from build123d import *

# Parameters (mm, degrees)
BOSS_EXTRUDE1_DEPTH = 10
SKETCH2_R           = 10
CUT_EXTRUDE1_DEPTH  = 140.306317158


with BuildPart() as part:
    # Sketch1 → Boss-Extrude1 (new body)
    with BuildSketch(Plane.XY):
        with BuildLine():
            Line((-117.5, 20), (117.5, 20))
            ThreePointArc((117.5, 20), (137.5, 0), (117.5, -20))
            Line((117.5, -20), (-117.5, -20))
            ThreePointArc((-117.5, -20), (-137.5, 0), (-117.5, 20))
        make_face()
    extrude(amount=BOSS_EXTRUDE1_DEPTH)

    # Sketch2 → Cut-Extrude1 (cut, through all)
    with BuildSketch(Plane.XY.offset(10)):
        with Locations((-117.5, 0)):
            Circle(SKETCH2_R)
        with Locations((117.5, 0)):
            Circle(SKETCH2_R)
    extrude(amount=-CUT_EXTRUDE1_DEPTH, mode=Mode.SUBTRACT)


solid = part.part
The model under review builds one solid part; all positions refer to its coordinate system, in mm. Give positions to 0.01 mm unless a question says otherwise; leave off trailing zeros. Order: outer loops, then holes, each group sorted by start corner. A loop starts at its lowest first (then second) coordinate and runs counter-clockwise, first axis right, second up. Notation, with made-up numbers: M 80.25,-19 L 114.25,-19 A32 cw 114.25,19 Z; hole C 3,-34 d5. An arc over 180 degrees is marked long. Answer in a Markdown table with one row per item. Add a question column.
1. Mouldability with a two-part tool opening along X and no side actions: class faces 1 (the cylindrical face through (107.51, 0.44, 5.07)), 2 (the cylindrical face through (137.495, 0.44, 4.93)), 3 (the flat face through (-2, 20, 5)) as released by +X, released by -X, zero draft, split by the parting line, or undercut.
2. Add section C-C on y = 13.5. State the section outline as (x, z) points, plus the area to 3 significant figures.
3. For pin 1 Ø1 at (y, z) = (13, 3.5) entering from -X; pin 2 Ø1.5 at (y, z) = (-13.5, 3) entering from -X, all flat-tipped, find the tip position at first contact; note any pin that passes through.
4. Add section B-B on z = 6.75. State the section outline as (x, y) points.
5. Add section A-A on y = 0. State the section outline as (x, z) points.
6. To check wall thickness, follow line 1 along X through (y, z) = (0.5, 5.25); line 2 along X through (y, z) = (1, 5.5); line 3 along Y through (x, z) = (117.5, 2.75). State the ranges of each line that lie inside material, in increasing order.
The answers:
| question | item | result |
|---|---|---|
| 1 | face 1 | undercut |
| 1 | face 2 | released by +X |
| 1 | face 3 | zero draft |
| 2 | outline | M -132.26,0 L 132.26,0 L 132.26,10 L -132.26,10 Z |
| 2 | area | 2,650 mm2 |
| 3 | pin 1 | x = -133.11 |
| 3 | pin 2 | x = -132.91 |
| 4 | outline | M -117.5,-20 L 117.5,-20 A20 ccw 117.5,20 L -117.5,20 A20 ccw Z; hole C -117.5,0 d20; hole C 117.5,0 d20 |
| 5 | outline | M -137.5,0 L -127.5,0 L -127.5,10 L -137.5,10 Z; M -107.5,0 L 107.5,0 L 107.5,10 L -107.5,10 Z; M 127.5,0 L 137.5,0 L 137.5,10 L 127.5,10 Z |
| 6 | line 1 | -137.49 to -127.49, -107.51 to 107.51, 127.49 to 137.49 |
| 6 | line 2 | -137.47 to -127.45, -107.55 to 107.55, 127.45 to 137.47 |
| 6 | line 3 | -20 to -10, 10 to 20 |
